The model under review builds one solid part; all positions refer to its coordinate system, in mm. A direction names the side the tool comes from. Round coordinates to 2 decimals unless told otherwise and drop trailing zeros. Write each loop counter-clockwise with the first axis right and the second up, starting at its lowest first coordinate (ties: lowest second). Pieces come first, ordered by that corner, then holes. Notation, with made-up numbers: (-17.75, -13.75) - (-13.75, -13.75) arc R16 ccw to (-13.75, -6.75) - close; hole circle Ø6 at (0, -25). An arc over 180 degrees is marked (long way). Write each question's results on one line, items separated by ' | '.
```python
from build123d import *

# Parameters (mm, degrees)
SKETCH1_R              = 66.5
SKETCH1_R_2            = 45
BOSS_EXTRUDE1_DEPTH    = 90
M10_TAPPED_HOLE1_D     = 8.5
M10_TAPPED_HOLE1_DEPTH = 66.499
M10_TAPPED_HOLE1_TIP   = 2.553657631
SKETCH4_R              = 12.5
CUT_EXTRUDE1_DEPTH     = 12
CHAMFER1_SIZE          = 2


with BuildPart() as part:
    # Sketch1 → Boss-Extrude1 (new, symmetric)
    with BuildSketch(Plane(origin=(0, 0, 0), x_dir=(0, 0, -1), z_dir=(1, 0, 0))):
        with Locations(Location((0, 0, 0), (0, 0, 180))):
            Circle(SKETCH1_R)
        with Locations(Location((0, 0, 0), (0, 0, 180))):
            Circle(SKETCH1_R_2, mode=Mode.SUBTRACT)
    extrude(amount=BOSS_EXTRUDE1_DEPTH, both=True)

    # M10 Tapped Hole1
    with Locations(Plane.XY.offset(66.5)):
        with Locations((0, 0)):
            Hole(M10_TAPPED_HOLE1_D / 2, depth=M10_TAPPED_HOLE1_DEPTH)
            with Locations((0, 0, -(M10_TAPPED_HOLE1_DEPTH + M10_TAPPED_HOLE1_TIP / 2))):  # 118° drill point
                Cone(0, M10_TAPPED_HOLE1_D / 2, M10_TAPPED_HOLE1_TIP, mode=Mode.SUBTRACT)

    # Sketch4 → Cut-Extrude1 (cut)
    with BuildSketch(Plane.XY.offset(66.5)):
        Circle(SKETCH4_R)
    extrude(amount=-CUT_EXTRUDE1_DEPTH, mode=Mode.SUBTRACT)

    # Chamfer1
    chamfer1_edges = [part.edges().sort_by_distance(p)[0] for p in [
        (-90, 0, -45),
        (90, 0, -45),
    ]]
    chamfer(chamfer1_edges, length=CHAMFER1_SIZE)


solid = part.part
```
Q1. For probe 1 along Y at (x, z) = (-7, 0); probe 2 along Y at (x, z) = (-17, 37); probe 3 along Z at (x, y) = (60, -25.5), list the stretches that pass through material, from the lowest coordinate up.
Evaluation:
probe 1: y = -66.5 to -45, 45 to 66.5 | probe 2: y = -55.26 to -25.61, 25.61 to 55.26 | probe 3: z = -61.42 to -37.08, 37.08 to 61.42
Q2. We need section C-C (x = -49). State the section outline as (y, z) points, plus the area to 3 significant figures.
Evaluation:
outline: circle Ø133 at (0, 0); hole circle Ø90 at (0, 0) | area: 7,530 mm^2
Q3. We need section D-D (x = 0). State the section outline as (y, z) points.
Evaluation:
outline: (-12.5, 54.5) - (-12.5, 65.31) arc R66.5 ccw (long way) to (12.5, 65.31) - (12.5, 54.5) - (4.25, 54.5) - (4.25, 44.8) arc R45 cw (long way) to (-4.25, 44.8) - (-4.25, 54.5) - close
Q4. We need section B-B (z = 0). State the section outline as (x, y) points, plus the area to 3 significant figures.
Evaluation:
outline: (-90, -66.5) - (90, -66.5) - (90, -47) - (88, -45) - (-88, -45) - (-90, -47) - close; (-90, 47) - (-88, 45) - (88, 45) - (90, 47) - (90, 66.5) - (-90, 66.5) - close | area: 7,730 mm^2
Q5. Tool access review of faces 5 (the cylindrical face through (-2.285, 3.584, 49.582)), 6 (the cylindrical face through (-1.232, 39.923, 20.765)): name each direction out of +Z, -Z, +X, -X, +Y, -Y from which nothing blocks a thin tool from reaching the whole face with its end or side.
Evaluation:
face 5: +Z | face 6: +X, -X
Q6. We need section A-A (y = 0). State the section outline as (x, z) points, plus the area to 3 significant figures.
Evaluation:
outline: (-90, -66.5) - (90, -66.5) - (90, -47) - (88, -45) - (-88, -45) - (-90, -47) - close; (-90, 47) - (-88, 45) - (-4.25, 45) - (-4.25, 54.5) - (-12.5, 54.5) - (-12.5, 66.5) - (-90, 66.5) - close; (4.25, 45) - (88, 45) - (90, 47) - (90, 66.5) - (12.5, 66.5) - (12.5, 54.5) - (4.25, 54.5) - close | area: 7,350 mm^2
Q7. The part is to be moulded in two halves that separate along Y. For faces 1 (the cylindrical face through (-12.488, 0.55, 60.584)), 2 (the flat face through (-90, 13.8, -45.3)), 3 (the flat face through (0, -5, 54.5)), 4 (the cylindrical face through (1.26, -56.073, 35.75)), say which applies: released by +Y, released by -Y, zero draft, split by the parting line, or undercut.
Evaluation:
face 1: undercut | face 2: zero draft | face 3: undercut | face 4: split by the parting line
Q8. Insertion check: P1, Ø12, axis at x = -43.5, z = 20.5, coming from the -Y side; P2, Ø4, axis at x = 20, z = -7.5, coming from the -Y side; P3, Ø1, axis at x = -19, y = 51.5, coming from the +Z side. Each pin has a flat end and moves straight along its axis. Give the tip position at first contact, or say it passes through.
Evaluation:
P1: stops at y = -64.9 | P2: stops at y = -66.27 | P3: stops at z = 42.68
